```python
from build123d import *

# Parameters (mm, degrees)
SKETCH1_R            = 42.5
SKETCH1_R_2          = 20
BOSS_EXTRUDE1_DEPTH  = 20
M6_CLEARANCE_HOLE1_D = 7
SKETCH4_R            = 26
CUT_EXTRUDE1_DEPTH   = 15
SKETCH5_R            = 29
SKETCH5_R_2          = 26.75
BOSS_EXTRUDE3_DEPTH  = 2
CUT_EXTRUDE2_START   = -12
SKETCH6_R            = 26.75
CUT_EXTRUDE2_DEPTH   = 12
SKETCH7_R            = 5.5
CUT_EXTRUDE3_DEPTH   = 7


with BuildPart() as part:
    # Sketch1 → Boss-Extrude1 (new body)
    with BuildSketch(Plane.XZ):
        with Locations(Location((0, 0, 0), (0, 0, 270))):
            Circle(SKETCH1_R)
        with Locations(Location((0, 0, 0), (0, 0, 270))):
            Circle(SKETCH1_R_2, mode=Mode.SUBTRACT)
    extrude(amount=BOSS_EXTRUDE1_DEPTH)

    # M6 Clearance Hole1 (through all)
    with Locations(Plane(origin=(0, 0, 0), x_dir=(1, 0, 0), z_dir=(0, 1, 0))):
        with Locations((0, -35), (0, 35), (-35, 0), (35, 0)):
            Hole(M6_CLEARANCE_HOLE1_D / 2)

    # Sketch4 → Cut-Extrude1 (cut)
    with BuildSketch(Plane(origin=(0, 0, 0), x_dir=(1, 0, 0), z_dir=(0, 1, 0))):
        with Locations(Location((0, 0, 0), (0, 0, 270))):
            Circle(SKETCH4_R)
    extrude(amount=-CUT_EXTRUDE1_DEPTH, mode=Mode.SUBTRACT)

    # Sketch5 → Boss-Extrude3 (add)
    with BuildSketch(Plane(origin=(0, 0, 0), x_dir=(1, 0, 0), z_dir=(0, 1, 0))):
        with Locations(Location((0, 0, 0), (0, 0, 90))):
            Circle(SKETCH5_R)
        with Locations(Location((0, 0, 0), (0, 0, 270))):
            Circle(SKETCH5_R_2, mode=Mode.SUBTRACT)
    extrude(amount=BOSS_EXTRUDE3_DEPTH)

    # Sketch6 → Cut-Extrude2 (cut)
    with BuildSketch(Plane(origin=(0, 2, 0), x_dir=(1, 0, 0), z_dir=(0, 1, 0)).offset(CUT_EXTRUDE2_START)):
        with Locations(Location((0, 0, 0), (0, 0, 270))):
            Circle(SKETCH6_R)
    extrude(amount=CUT_EXTRUDE2_DEPTH, mode=Mode.SUBTRACT)

    # Sketch7 → Cut-Extrude3 (cut)
    with BuildSketch(Plane.XZ.offset(20)):
        with Locations(Location((0, 35, 0), (0, 0, 270))):
            Circle(SKETCH7_R)
        with Locations(Location((-35, 0, 0), (0, 0, 270))):
            Circle(SKETCH7_R)
        with Locations(Location((0, -35, 0), (0, 0, 270))):
            Circle(SKETCH7_R)
        with Locations(Location((35, 0, 0), (0, 0, 270))):
            Circle(SKETCH7_R)
    extrude(amount=-CUT_EXTRUDE3_DEPTH, mode=Mode.SUBTRACT)


solid = part.part
```
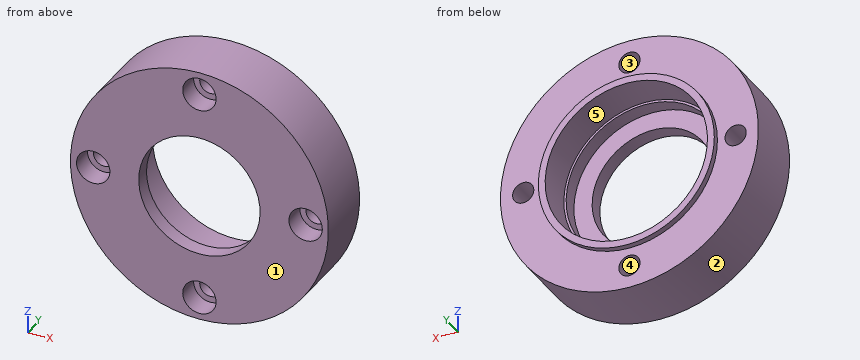
Could you check a few things on this model? Use its own coordinates, in mm. Face numbers are marked on the shaded views. A direction names the side the tool comes from. Coordinates: 2 decimals unless noted, no trailing zeros. Write each loop counter-clockwise with the first axis right and the second up, starting at its lowest first coordinate (ties: lowest second). Pieces come first, ordered by that corner, then holes. Notation, with made-up numbers: (57.25, 36.25) - (85.25, 36.25) arc R20 ccw to (85.25, 59.25) - close; hole circle Ø4 at (33, 48.5). An arc over 180 degrees is marked (long way). Use a Markdown table: item, result.
Q1. I'm going to push flat-ended pins straight in: pin 1 Ø12 at (x, y) = (14.5, -16.5) entering from +Z; pin 2 Ø2 at (x, y) = (-22, -3.5) entering from -Z; pin 3 Ø1.5 at (y, z) = (-1, 22) entering from -X; pin 4 Ø24 at (x, z) = (0, 0) entering from -Y. Where does each tip first touch, or does it pass through?
Geometry check:
| item | result |
|---|---|
| pin 1 | stops at z = 41.64 |
| pin 2 | stops at z = -36.95 |
| pin 3 | stops at x = -36.81 |
| pin 4 | passes through |
Q2. Imagine slicing it at D-D (x = 28). List the corners of the cut face in (y, z) for me, and give its area (3 significant figures).
Geometry check:
| item | result |
|---|---|
| outline | (-20, -31.97) - (0, -31.97) - (0, -7.55) - (2, -7.55) - (2, 7.55) - (0, 7.55) - (0, 31.97) - (-20, 31.97) - close |
| area | 1,310 mm2 |
Q3. Thinking about a two-plate mould opening in Z: for the marked faces 1, 2 and 3, which applies, +Z half, -Z half, draft (parallel to the pull), parting line (faces both ways), or undercut?
Geometry check:
| item | result |
|---|---|
| face 1 | draft |
| face 2 | parting line |
| face 3 | undercut |
Q4. Please list where these lines run through material, in increasing order: L1, parallel to X at y = -13.85, z = 0; L2, parallel to Z at x = 2.5, y = -4.25; L3, parallel to Y at x = 37, z = -13.5.
Geometry check:
| item | result |
|---|---|
| L1 | x = -42.5 to -40.5, -29.5 to -26, 26 to 29.5, 40.5 to 42.5 |
| L2 | z = -42.43 to -37.45, -32.55 to -26.63, 26.63 to 32.55, 37.45 to 42.43 |
| L3 | y = -20 to 0 |
Q5. Imagine slicing it at A-A (x = 11). List the corners of the cut face in (y, z) for me, and give its area (3 significant figures).
Geometry check:
| item | result |
|---|---|
| outline | (-20, -41.05) - (0, -41.05) - (0, -26.83) - (2, -26.83) - (2, -24.38) - (-10, -24.38) - (-10, -23.56) - (-15, -23.56) - (-15, -16.7) - (-20, -16.7) - close; (-20, 16.7) - (-15, 16.7) - (-15, 23.56) - (-10, 23.56) - (-10, 24.38) - (2, 24.38) - (2, 26.83) - (0, 26.83) - (0, 41.05) - (-20, 41.05) - close |
| area | 762 mm2 |
Q6. Imagine slicing it at C-C (z = 4.5). List the corners of the cut face in (x, y) for me, and give its area (3 significant figures).
Geometry check:
| item | result |
|---|---|
| outline | (-42.26, -20) - (-38.16, -20) - (-38.16, -13) - (-31.84, -13) - (-31.84, -20) - (-19.49, -20) - (-19.49, -15) - (-25.61, -15) - (-25.61, -10) - (-26.37, -10) - (-26.37, 2) - (-28.65, 2) - (-28.65, 0) - (-42.26, 0) - close; (19.49, -20) - (31.84, -20) - (31.84, -13) - (38.16, -13) - (38.16, -20) - (42.26, -20) - (42.26, 0) - (28.65, 0) - (28.65, 2) - (26.37, 2) - (26.37, -10) - (25.61, -10) - (25.61, -15) - (19.49, -15) - close |
| area | 633 mm2 |
Q7. Imagine slicing it at B-B (y = -8.25). List the corners of the cut face in (x, z) for me.
Geometry check:
| item | result |
|---|---|
| outline | circle Ø85 at (0, 0); hole circle Ø7 at (-35, 0); hole circle Ø53.5 at (0, 0); hole circle Ø7 at (0, -35); hole circle Ø7 at (0, 35); hole circle Ø7 at (35, 0) |
Q8. Which directions (+Z, -Z, +X, -X, +Y, -Y) give clear straight access to the entire face, cutting with the end or side of a thin tool? Please do the marked faces 4 and 5.
Geometry check:
| item | result |
|---|---|
| face 4 | +Y, -Y |
| face 5 | +Y |
